from build123d import *

# Parameters (mm, degrees)
SKETCH_2_R          = 11
EXTRUDE_1_DEPTH     = 5
SKETCH_3_R          = 9
CUT_EXTRUDE_1_DEPTH = 5
CHAMFER_2_SIZE      = 0.3


with BuildPart() as part:
    # 草图2 → 凸台-拉伸1 (new body)
    with BuildSketch(Plane.XY):
        Circle(SKETCH_2_R)
    extrude(amount=EXTRUDE_1_DEPTH)

    # 草图3 → 切除-拉伸1 (cut)
    with BuildSketch(Plane.XY.offset(5)):
        Circle(SKETCH_3_R)
    extrude(amount=-CUT_EXTRUDE_1_DEPTH, mode=Mode.SUBTRACT)

    # 倒角2
    chamfer_2_edges = [part.edges().sort_by_distance(p)[0] for p in [
        (-11, 0, 0),
        (-11, 0, 5),
        (-9, 0, 0),
        (-9, 0, 5),
    ]]
    chamfer(chamfer_2_edges, length=CHAMFER_2_SIZE)


solid = part.part
Here's how the part is built. I have some questions about the finished solid (model axes, mm). Give positions to 0.01 mm unless a question says otherwise; leave off trailing zeros. Loops run counter-clockwise (first coordinate to the right, second up) from the corner with the lowest first, then second, coordinate; pieces in that order, holes last. Notation, with made-up numbers: (69, 2) -> (100, 2) arc R11 ccw to (100, 22) -> close; hole circle Ø7 at (62.25, 39). An arc over 180 degrees is marked (long way). Answer as a JSON object with one key per item and string values. Group by question number.
Item 1: Thinking about a two-plate mould opening in X: for faces 1 (the cylindrical face through (-2.38, -10.74, 2.47)), 2 (the flat face through (-3, 9, 0)), 3 (the cylindrical face through (-1.172, 8.923, 2.531)), which applies, pulls with the +X half, pulls with the -X half, needs draft (parallel to the pull), parting line crosses it, or undercut?
Item 2: Imagine slicing it at C-C on z = 0.75. Write out the boundary of the cut face in (x, y).
Item 3: I need wall thicknesses on L1, parallel to Y at x = 0, z = 3.65; L2, parallel to X at y = -8, z = 0.65; L3, parallel to X at y = -2, z = 3.15. Which ranges of each line are inside material? Lowest first, please.
Item 4: Imagine slicing it at A-A on x = 0. Write out the boundary of the cut face in (y, z), then the cut area to 3 significant figures.
Item 5: Will these pins go through, and if not, where does the flat tip stop? pin 1 (1 mm diameter, centred on y = -2.5, z = 2.5, fed in from +X); pin 2 (3 mm diameter, centred on x = -7.5, z = 4.5, fed in from +Y); pin 3 (2 mm diameter, centred on y = 8, z = 2.5, fed in from -X).
Answer list:
{
 "1": {"face 1": "parting line crosses it", "face 2": "needs draft", "face 3": "undercut"},
 "2": {"outline": "circle Ø22 at (0, 0); hole circle Ø18 at (0, 0)"},
 "3": {"L1": "y = -11 to -9, 9 to 11", "L2": "x = -7.55 to -4.12, 4.12 to 7.55", "L3": "x = -10.82 to -8.77, 8.77 to 10.82"},
 "4": {"outline": "(-11, 0.3) -> (-10.7, 0) -> (-9.3, 0) -> (-9, 0.3) -> (-9, 4.7) -> (-9.3, 5) -> (-10.7, 5) -> (-11, 4.7) -> close; (9, 0.3) -> (9.3, 0) -> (10.7, 0) -> (11, 0.3) -> (11, 4.7) -> (10.7, 5) -> (9.3, 5) -> (9, 4.7) -> close", "area": "19.6 mm2"},
 "5": {"pin 1": "stops at x = 10.82", "pin 2": "stops at y = 9.22", "pin 3": "stops at x = -8.49"}
}
